```python
from build123d import *

# Parameters (mm, degrees)
SKETCH_1_W          = 46
SKETCH_1_H          = 32
EXTRUDE_1_DEPTH     = 25.2
SKETCH_2_R          = 3.7
SKETCH_2_R_2        = 5
EXTRUDE_2_DEPTH     = 2
SKETCH_3_R          = 1.3
CUT_EXTRUDE_1_DEPTH = 10
SKETCH_4_R          = 4
EXTRUDE_3_DEPTH     = 19
CUT_EXTRUDE_START   = -16
CUT_EXTRUDE_2_DEPTH = 16
SKETCH_6_R          = 12.1
EXTRUDE_4_DEPTH     = 31
EXTRUDE_5_DEPTH     = 4
CUT_EXTRUDE_3_DEPTH = 88.342884876


with BuildPart() as part:
    # 草图1 → 凸台-拉伸1 (new body)
    with BuildSketch(Plane.XY):
        with Locations((23, 16)):
            Rectangle(SKETCH_1_W, SKETCH_1_H)
    extrude(amount=EXTRUDE_1_DEPTH)

    # 草图2 → 凸台-拉伸2 (add)
    with BuildSketch(Plane.XY.offset(25.2)):
        with Locations(Location((6, 25, 0), (0, 0, 180))):
            Circle(SKETCH_2_R)
        with Locations(Location((6, 7, 0), (0, 0, 180))):
            Circle(SKETCH_2_R)
        with Locations(Location((39, 7, 0), (0, 0, 180))):
            Circle(SKETCH_2_R)
        with Locations(Location((39, 25, 0), (0, 0, 180))):
            Circle(SKETCH_2_R)
        with Locations(Location((15, 16, 0), (0, 0, 180))):
            Circle(SKETCH_2_R_2)
    extrude(amount=EXTRUDE_2_DEPTH)

    # 草图3 → 切除-拉伸1 (cut)
    with BuildSketch(Plane.XY.offset(27.2)):
        with Locations((6, 7)):
            Circle(SKETCH_3_R)
        with Locations((6, 25)):
            Circle(SKETCH_3_R)
        with Locations((39, 25)):
            Circle(SKETCH_3_R)
        with Locations((39, 7)):
            Circle(SKETCH_3_R)
    extrude(amount=-CUT_EXTRUDE_1_DEPTH, mode=Mode.SUBTRACT)

    # 草图4 → 凸台-拉伸3 (add)
    with BuildSketch(Plane.XY.offset(27.2)):
        with Locations((15, 16)):
            Circle(SKETCH_4_R)
    extrude(amount=EXTRUDE_3_DEPTH)

    # 草图5 → 切除-拉伸2 (cut)
    with BuildSketch(Plane.XY.offset(46.2).offset(CUT_EXTRUDE_START)):
        with BuildLine():
            Line((17.107130751, 19.4), (12.892869249, 19.4))
            ThreePointArc((12.892869249, 19.4), (15, 20), (17.107130751, 19.4))
        make_face()
    extrude(amount=CUT_EXTRUDE_2_DEPTH, mode=Mode.SUBTRACT)

    # 草图6 → 凸台-拉伸4 (add)
    with BuildSketch(Plane(origin=(46, 0, 0), x_dir=(0, 0, -1), z_dir=(1, 0, 0))):
        with Locations(Location((-11.1, 19.9, 0), (0, 0, 90))):
            Circle(SKETCH_6_R)
    extrude(amount=EXTRUDE_4_DEPTH)

    # 草图7 → 凸台-拉伸5 (add)
    with BuildSketch(Plane(origin=(77, 0, 0), x_dir=(0, 0, -1), z_dir=(1, 0, 0))):
        Polygon((-19.231728338, 25.910407286), (-17.110407994, 28.03172763), (-16.403301178, 27.324620884), (-18.524621557, 25.203300505), align=None)
        Polygon((-5.796699495, 12.475378443), (-3.675379152, 14.596698787), (-2.96827237, 13.889592006), (-5.089592714, 11.768271662), align=None)
    extrude(amount=EXTRUDE_5_DEPTH)

    # 草图8 → 切除-拉伸3 (cut, through all)
    with BuildSketch(Plane(origin=(0, 22.571067812, 22.571067812), x_dir=(1, 0, 0), z_dir=(0, 0.7071067811865464, 0.7071067811865487))):
        with BuildLine():
            Line((77.969259397, 6.842291957), (79.821949512, 6.842291957))
            ThreePointArc((79.821949512, 6.842291957), (80.341395338, 6.32284613), (79.821949512, 5.803400304))
            Line((79.821949512, 5.803400304), (77.969259397, 5.803400304))
            ThreePointArc((77.969259397, 5.803400304), (77.44981357, 6.32284613), (77.969259397, 6.842291957))
        make_face()
    extrude(amount=-CUT_EXTRUDE_3_DEPTH, mode=Mode.SUBTRACT)


solid = part.part
```
Verification items for the finished model (mm, model axes). A direction names the side the tool comes from. Round coordinates to 2 decimals unless told otherwise and drop trailing zeros. Order: outer loops, then holes, each group sorted by start corner. A loop starts at its lowest first (then second) coordinate and runs counter-clockwise, first axis right, second up. Notation, with made-up numbers: (22.25, 43.5) -> (68.25, 43.5) arc R12 cw to (68.25, 49.5) -> close; hole circle Ø10 at (55.25, 83). An arc over 180 degrees is marked (long way). Put each result on its own line as item: value. Start each with the question number.
(1) Draft check along X on faces 4 (the face through (4.29, 28.28, 26.19)), 5 (the face through (46, 9, 18)), 6 (the face through (78.97, 13.05, 5.22)). Enter one of: +X half, -X half, draft (parallel to the pull), parting line (faces both ways), or undercut.
(2) Depth check by flat-ended pin: pin 1 Ø2 at (y, z) = (29.5, 5) entering from +X; pin 2 Ø10 at (x, y) = (42.5, 8) entering from +Z; pin 3 Ø4 at (x, y) = (55, 7.5) entering from -Z. Enter the tip coordinate at first touch or a pass-through.
(3) Section check B-B (x = 15). Enter the section's corners in (y, z), then the cut area to 3 significant figures.
(4) Section check A-A (y = 7). Enter the section's corners in (x, z).
(5) Section check C-C (x = 39). Enter the section's corners in (y, z).
(6) Section check D-D (y = 16). Enter the section's corners in (x, z), then the cut area to 3 significant figures.
(7) Tool access check on faces 1 (the face through (61.283, 31.441, 14.735)), 2 (the face through (14.133, 12.095, 36.567)), 3 (the face through (78.97, 12.37, 4.49)). Record the directions out of +Z, -Z, +X, -X, +Y, -Y that give a thin tool (end or side, any length) a straight path to the whole face; none if there is none.
(8) Material ranges on line 1 along Y through (x, z) = (6, 21); line 2 along Z through (x, y) = (5.5, 7.5); line 3 along Z through (x, y) = (45.5, 27), recorded low to high.
Completed:
1. face 4: undercut
1. face 5: +X half
1. face 6: draft
2. pin 1: stops at x = 77
2. pin 2: stops at z = 27.2
2. pin 3: stops at z = 4.92
3. outline: (0, 0) -> (32, 0) -> (32, 25.2) -> (21, 25.2) -> (21, 27.2) -> (20, 27.2) -> (20, 30.2) -> (19.4, 30.2) -> (19.4, 46.2) -> (12, 46.2) -> (12, 27.2) -> (11, 27.2) -> (11, 25.2) -> (0, 25.2) -> close
3. area: 969 mm2
4. outline: (0, 0) -> (46, 0) -> (46, 25.2) -> (42.7, 25.2) -> (42.7, 27.2) -> (40.3, 27.2) -> (40.3, 17.2) -> (37.7, 17.2) -> (37.7, 27.2) -> (35.3, 27.2) -> (35.3, 25.2) -> (9.7, 25.2) -> (9.7, 27.2) -> (7.3, 27.2) -> (7.3, 17.2) -> (4.7, 17.2) -> (4.7, 27.2) -> (2.3, 27.2) -> (2.3, 25.2) -> (0, 25.2) -> close
5. outline: (0, 0) -> (32, 0) -> (32, 25.2) -> (28.7, 25.2) -> (28.7, 27.2) -> (26.3, 27.2) -> (26.3, 17.2) -> (23.7, 17.2) -> (23.7, 27.2) -> (21.3, 27.2) -> (21.3, 25.2) -> (10.7, 25.2) -> (10.7, 27.2) -> (8.3, 27.2) -> (8.3, 17.2) -> (5.7, 17.2) -> (5.7, 27.2) -> (3.3, 27.2) -> (3.3, 25.2) -> (0, 25.2) -> close
6. outline: (0, 0) -> (46, 0) -> (46, -0.35) -> (77, -0.35) -> (77, 22.55) -> (46, 22.55) -> (46, 25.2) -> (20, 25.2) -> (20, 27.2) -> (19, 27.2) -> (19, 46.2) -> (11, 46.2) -> (11, 27.2) -> (10, 27.2) -> (10, 25.2) -> (0, 25.2) -> close
6. area: 2,040 mm2
7. face 1: +X
7. face 2: +Z
7. face 3: -Z, +X, -Y
8. line 1: y = 0 to 5.7, 8.3 to 23.7, 26.3 to 32
8. line 2: z = 0 to 17.2
8. line 3: z = 0 to 25.2
